```python
from build123d import *

# Parameters (mm, degrees)
SKETCH1_R      = 9
SKETCH1_R_2    = 10
SKETCH1_R_3    = 20
EXTRUDE1_DEPTH = 20
FILLET1_R      = 3
FILLET2_R      = 10
CHAMFER1_SIZE  = 2.5


with BuildPart() as part:
    # Sketch1 → Extrude1 (new body)
    with BuildSketch(Plane.XY):
        with BuildLine():
            Line((-54.5, 278), (-62, 320))
            Line((-62, 320), (-27.139905674, 323.126311493))
            Line((-27.139905674, 323.126311493), (12.815444518, 390.231864585))
            ThreePointArc((12.815444518, 390.231864585), (35.306076251, 399.283297302), (50, 380))
            Line((50, 380), (50, 0))
            ThreePointArc((50, 0), (0, -50), (-50, 0))
            Line((-50, 0), (-50, 90))
            ThreePointArc((-50, 90), (-17.234137889, 181.62959318), (-17.807748235, 278.939690485))
            ThreePointArc((-17.807748235, 278.939690485), (-21.406992079, 284.267795368), (-27.765067315, 285.22599012))
            Line((-27.765067315, 285.22599012), (-54.5, 278))
        make_face()
        with Locations((0, 60)):
            Circle(SKETCH1_R, mode=Mode.SUBTRACT)
        with Locations((30, 380)):
            Circle(SKETCH1_R_2, mode=Mode.SUBTRACT)
        Circle(SKETCH1_R_3, mode=Mode.SUBTRACT)
    extrude(amount=EXTRUDE1_DEPTH)

    # Fillet1
    fillet1_edges = [part.edges().sort_by_distance(p)[0] for p in [
        (-54.5, 278, 10),
        (-62, 320, 10),
    ]]
    fillet(fillet1_edges, radius=FILLET1_R)

    # Fillet2
    fillet2_edges = [part.edges().sort_by_distance(p)[0] for p in [
        (-27.139905674, 323.126311493, 10),
    ]]
    fillet(fillet2_edges, radius=FILLET2_R)

    # Chamfer1
    chamfer1_edges = [part.edges().sort_by_distance(p)[0] for p in [
        (-20, 0, 0),
    ]]
    chamfer(chamfer1_edges, length=CHAMFER1_SIZE)


solid = part.part
```
CAD build for the part. Positions are in the model's coordinates, mm. A direction names the side the tool comes from. Give positions to 0.01 mm unless a question says otherwise; leave off trailing zeros. Order: outer loops, then holes, each group sorted by start corner. A loop starts at its lowest first (then second) coordinate and runs counter-clockwise, first axis right, second up.
(1) Mould opens along Y. For faces 4 (the flat face through (-39.387, 282.085, 9.86)), 5 (the flat face through (-6.12, 358.43, 9.86)), 6 (the cylindrical face through (1.099, -49.988, 9.86)) say: released by +Y, released by -Y, zero draft, split by the parting line, or undercut.
(2) Saw through at C-C, the plane z = 11.5. Give the cut face in (x, y), then the cut area to 3 significant figures.
(3) Saw through at D-D, the plane x = 0. Give the cut face in (y, z), then the cut area to 3 significant figures.
(4) Tool access for faces 1 (the flat face through (-50, 44, 10)), 2 (the flat face through (7, 178, 0)), 3 (the cylindrical face through (-21.3, 284.2, 9.9)): list every direction of +Z, -Z, +X, -X, +Y, -Y with a clear straight run to the whole face (end or side of a thin tool).
(5) Flat gauge pins, fed straight in: pin 1 (14.5 mm diameter, centred on x = 0, y = 60, fed in from -Z); pin 2 (2 mm diameter, centred on x = -25, z = 5, fed in from +Y); pin 3 (1.5 mm diameter, centred on x = 7.5, z = 2, fed in from -Y); pin 4 (12 mm diameter, centred on x = -20.5, z = 8, fed in from -Y). Where does each tip first touch, or does it go through?
(6) Saw through at A-A, the plane x = 30. Give the cut face in (y, z).
(7) Saw through at B-B, the plane y = 60. Give the cut face in (x, z).
(8) Drill centre lines: L1, parallel to Y at x = 0, z = 11.5; L2, parallel to Y at x = 0.5, z = 3; L3, parallel to X at y = 31, z = 9.75. Where is each one in solid material? Low to high.
Results found:
1. face 4: undercut
1. face 5: released by +Y
1. face 6: released by -Y
2. outline: (-61.42, 316.78) - (-55.08, 281.22) arc R3 ccw to (-51.34, 278.85) - (-27.77, 285.23) arc R8 cw to (-17.81, 278.94) arc R280 cw to (-50, 90) - (-50, 0) arc R50 ccw to (50, 0) - (50, 380) arc R20 ccw to (12.82, 390.23) - (-24.53, 327.51) arc R10 cw to (-32.23, 322.67) - (-58.74, 320.29) arc R3 ccw to start; hole circle Ø40 at (0, 0); hole circle Ø18 at (0, 60); hole circle Ø20 at (30, 380)
2. area: 33,500 mm2
3. outline: (-50, 0) - (-22.5, 0) - (-20, 2.5) - (-20, 20) - (-50, 20) - close; (20, 2.5) - (22.5, 0) - (51, 0) - (51, 20) - (20, 20) - close; (69, 0) - (368.71, 0) - (368.71, 20) - (69, 20) - close
3. area: 7,210 mm2
4. face 1: +Z, -Z, -X, -Y
4. face 2: -Z, +X, -X, +Y, -Y
4. face 3: +Z, -Z
5. pin 1: passes through
5. pin 2: stops at y = 328.4
5. pin 3: stops at y = -49.54
5. pin 4: stops at y = -47.85
6. outline: (-40, 0) - (370, 0) - (370, 20) - (-40, 20) - close; (390, 0) - (400, 0) - (400, 20) - (390, 20) - close
7. outline: (-50, 0) - (-9, 0) - (-9, 20) - (-50, 20) - close; (9, 0) - (50, 0) - (50, 20) - (9, 20) - close
8. L1: y = -50 to -20, 20 to 51, 69 to 368.71
8. L2: y = -50 to -19.99, 19.99 to 51.01, 68.99 to 369.55
8. L3: x = -50 to 50
